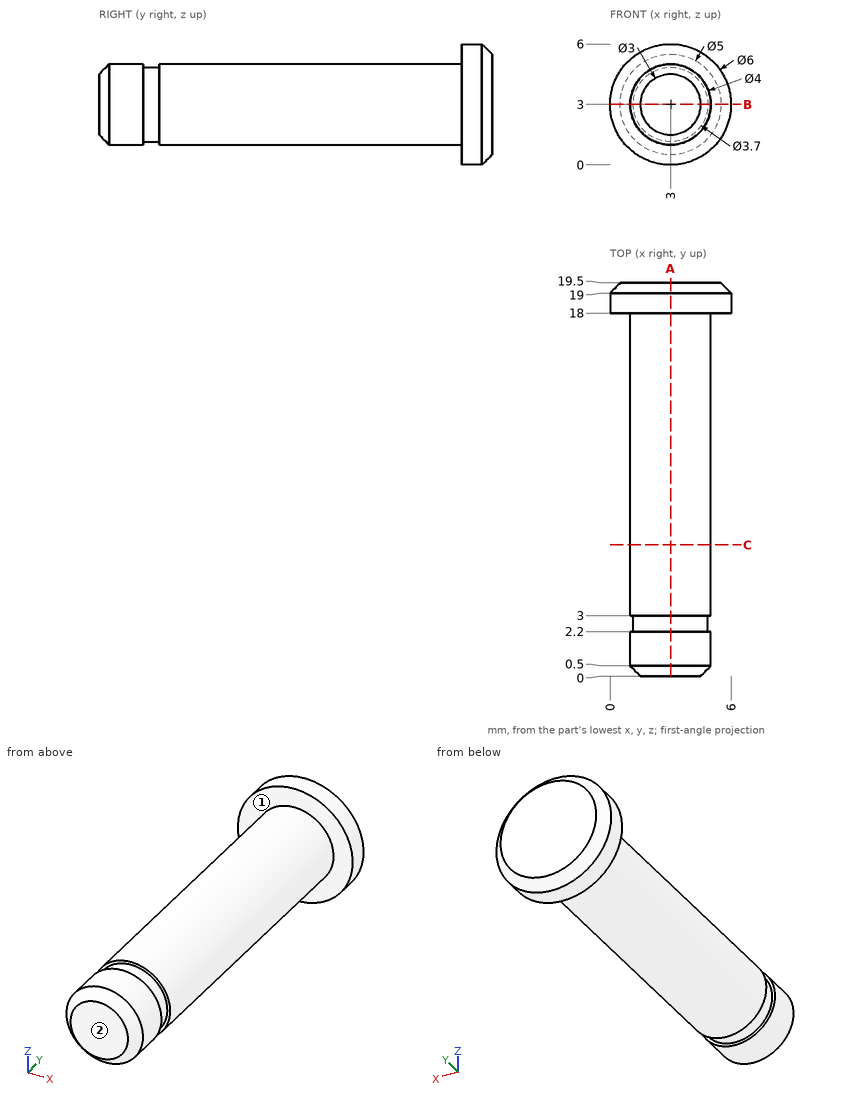
Study the drawing (mm; zero at the part's minimum x, y, z) and answer. A direction names the side the tool comes from. Give positions to 0.01 mm unless a question says otherwise; leave off trailing zeros. Order: outer loops, then holes, each group sorted by start corner. A loop starts at its lowest first (then second) coordinate and runs counter-clockwise, first axis right, second up.
1. Section B-B, the plane z = 3 is taken. Determine the outline of the cut face in (x, y).
Result sheet:
outline: (0, 18) - (1, 18) - (1, 3) - (1.15, 3) - (1.15, 2.2) - (1, 2.2) - (1, 0.5) - (1.5, 0) - (4.5, 0) - (5, 0.5) - (5, 2.2) - (4.85, 2.2) - (4.85, 3) - (5, 3) - (5, 18) - (6, 18) - (6, 19) - (5.5, 19.5) - (0.5, 19.5) - (0, 19) - close
2. Section C-C, the plane y = 6.5 is taken. Determine the outline of the cut face in (x, z), and give its area (3 significant figures).
Result sheet:
outline: circle Ø4 at (3, 3)
area: 12.6 mm2
3. Straight lines are drawn through the part: L1, parallel to Y at x = 4, z = 5.15; L2, parallel to Z at x = 1.25, y = 14.25; L3, parallel to Y at x = 4.6, z = 2.45. For each, find the intervals that lie inside material, in ascending order.
Result sheet:
L1: y = 18 to 19.5
L2: z = 2.03 to 3.97
L3: y = 0.19 to 19.5
4. Section A-A, the plane x = 3 is taken. Determine the outline of the cut face in (y, z).
Result sheet:
outline: (0, 1.5) - (0.5, 1) - (2.2, 1) - (2.2, 1.15) - (3, 1.15) - (3, 1) - (18, 1) - (18, 0) - (19, 0) - (19.5, 0.5) - (19.5, 5.5) - (19, 6) - (18, 6) - (18, 5) - (3, 5) - (3, 4.85) - (2.2, 4.85) - (2.2, 5) - (0.5, 5) - (0, 4.5) - close
5. For the marked faces 1 and 2, determine the directions among +Z, -Z, +X, -X, +Y, -Y from which every point of the face is accessible in a straight line to the end or side of a thin tool.
Result sheet:
face 1: -Y
face 2: +Z, -Z, +X, -X, -Y
6. Each of these flat-tipped pins is pushed along its axis until it touches: P1, Ø1, axis at y = 10.5, z = 1, coming from the -X side; P2, Ø1, axis at y = 8.5, z = 3.5, coming from the -X side; P3, Ø1.5, axis at y = 14, z = 2.5, coming from the +X side. Where does it stop, or does it pass through?
Result sheet:
P1: stops at x = 1.68
P2: stops at x = 1
P3: stops at x = 5
